```python
from build123d import *

# Parameters (mm, degrees)
SKETCH1_W            = 260
SKETCH1_H            = 300
BOSS_EXTRUDE1_DEPTH  = 30
M12_THREADED_HOLE1_D = 10.2


with BuildPart() as part:
    # Sketch1 → Boss-Extrude1 (new body)
    with BuildSketch(Plane.XY):
        with Locations((130, 150)):
            Rectangle(SKETCH1_W, SKETCH1_H)
        with BuildLine():
            Line((115, 152), (145, 152))
            ThreePointArc((145, 152), (175, 122), (145, 92))
            Line((145, 92), (115, 92))
            ThreePointArc((115, 92), (85, 122), (115, 152))
        make_face(mode=Mode.SUBTRACT)
    extrude(amount=BOSS_EXTRUDE1_DEPTH)

    # M12 Threaded hole1 (through all)
    with Locations(Plane(origin=(50, 122, 30), x_dir=(1, 0, 0), z_dir=(0, 0, 1))):
        with Locations((0, 0), (160, 0)):
            Hole(M12_THREADED_HOLE1_D / 2)


solid = part.part
```
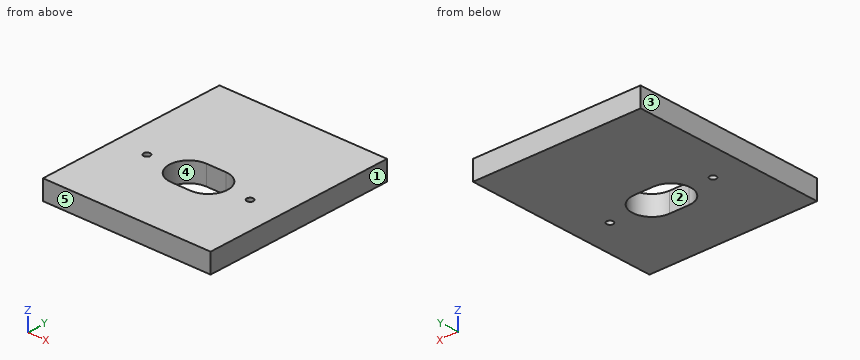
Work out the finished part from the listing and answer in its coordinate system (mm). Face numbers are marked on the shaded views. A direction names the side the tool comes from. Coordinates: 2 decimals unless noted, no trailing zeros. Order: outer loops, then holes, each group sorted by start corner. A loop starts at its lowest first (then second) coordinate and runs counter-clockwise, first axis right, second up. Notation, with made-up numbers: (39.5, 85.25) - (65.5, 85.25) arc R14 cw to (65.5, 95.25) - close; hole circle Ø7 at (70, -2). An arc over 180 degrees is marked (long way). Answer as a JSON object with one key per item and string values.
1. Find section B-B on z = 9.25. Determine the outline of the cut face in (x, y).
Output values:
{"outline": "(0, 0) - (260, 0) - (260, 300) - (0, 300) - close; hole circle Ø10.2 at (50, 122); hole (115, 92) - (145, 92) arc R30 ccw to (145, 152) - (115, 152) arc R30 ccw to start; hole circle Ø10.2 at (210, 122)"}
2. Find section D-D on x = 96. Determine the outline of the cut face in (y, z), plus the area to 3 significant figures.
Output values:
{"outline": "(0, 0) - (98.78, 0) - (98.78, 30) - (0, 30) - close; (145.22, 0) - (300, 0) - (300, 30) - (145.22, 30) - close", "area": "7,610 mm²"}
3. Consider line 1 (Y direction, x = 50, z = 21); line 2 (Y direction, x = 207.5, z = 24.5); line 3 (X direction, y = 116, z = 22.75). Determine where each line is inside the solid, lowest interval first.
Output values:
{"line 1": "y = 0 to 116.9, 127.1 to 300", "line 2": "y = 0 to 117.55, 126.45 to 300", "line 3": "x = 0 to 85.61, 174.39 to 260"}
4. Find section A-A on y = 122. Determine the outline of the cut face in (x, z), plus the area to 3 significant figures.
Output values:
{"outline": "(0, 0) - (44.9, 0) - (44.9, 30) - (0, 30) - close; (55.1, 0) - (85, 0) - (85, 30) - (55.1, 30) - close; (175, 0) - (204.9, 0) - (204.9, 30) - (175, 30) - close; (215.1, 0) - (260, 0) - (260, 30) - (215.1, 30) - close", "area": "4,490 mm²"}
5. A tool of negligible diameter and unlimited length cuts with its end or side. For the marked faces 1 and 2, from which of +Z, -Z, +X, -X, +Y, -Y can it reach the whole face along a straight path? Write none if from no direction.
Output values:
{"face 1": "+Z, -Z, +X, +Y, -Y", "face 2": "+Z, -Z"}
6. The mould has two halves that part along X. Classify the marked faces 3, 4 and 5: +X half, -X half, draft (parallel to the pull), parting line (faces both ways), or undercut.
Output values:
{"face 3": "-X half", "face 4": "undercut", "face 5": "draft"}
7. Find section C-C on x = 210. Determine the outline of the cut face in (y, z).
Output values:
{"outline": "(0, 0) - (116.9, 0) - (116.9, 30) - (0, 30) - close; (127.1, 0) - (300, 0) - (300, 30) - (127.1, 30) - close"}
